Part model, mm, in its own coordinate system. Face numbers are marked on the shaded views. A direction names the side the tool comes from. Round coordinates to 2 decimals unless told otherwise and drop trailing zeros. Write each loop counter-clockwise with the first axis right and the second up, starting at its lowest first coordinate (ties: lowest second). Pieces come first, ordered by that corner, then holes. Notation, with made-up numbers: (3, 43.25) -> (28, 43.25) arc R18 ccw to (28, 62.25) -> close; hole circle Ø9 at (21, 54). An arc over 180 degrees is marked (long way). Use CSV: the item, a comma, the result in double quotes. Start each with the question number.
(1) Saw through at D-D (y = -47.5). Give the cut face in (x, z), plus the area to 3 significant figures.
(2) Which spindle directions (+Z, -Z, +X, -X, +Y, -Y) get a long thin tool onto all of the face, cutting with end or side? Do the marked faces 4, 5 and 6. Say none if no direction does.
(3) Probe line 1 (Z direction, x = -31, y = -28.25); line 2 (Z direction, x = -33, y = -42); line 3 (Z direction, x = -31, y = -26.75). List the from-to ranges inside material, lowest first. Write a range as [from, to].
(4) Saw through at C-C (x = 13). Give the cut face in (y, z), plus the area to 3 significant figures.
(5) Saw through at B-B (z = -27.5). Give the cut face in (x, y).
(6) Two-plate mould, pull along Y, no slides. Class the marked faces 1, 2 and 3: released by +Y, released by -Y, zero draft, split by the parting line, or undercut.
(7) Saw through at A-A (y = -25). Give the cut face in (x, z), plus the area to 3 significant figures.
(8) Drop flat-ended pins along their axis: pin 1 (8 mm diameter, centred on y = -8.5, z = -2, fed in from -X); pin 2 (18.5 mm diameter, centred on x = 7.5, y = -34.5, fed in from -Z); pin 3 (11.5 mm diameter, centred on x = -20, z = -8.5, fed in from -Y). Give the stop position or say it passes through.
```python
from build123d import *

# Parameters (mm, degrees)
EXTRUDE_1_DEPTH        = 5
FILLET_1_R             = 3
CUT_EXTRUDE_1_REACH    = 77
SKETCH_2_R             = 19.5
SKETCH_4_W             = 10
SKETCH_4_H             = 30
EXTRUDE_2_DEPTH        = 30
CUT_EXTRUDE_3_REACH    = 105.024
HOLE_WIZARD_M6_1_D     = 5
HOLE_WIZARD_M6_1_DEPTH = 15
HOLE_WIZARD_M6_1_TIP   = 1.502151548
SKETCH_7_W             = 55
SKETCH_7_H             = 10
EXTRUDE_3_DEPTH        = 12


with BuildPart() as part:
    # 草图1 → 凸台-拉伸1 (new, symmetric)
    with BuildSketch(Plane.XY):
        Polygon((0, 0), (55, 0), (55, -50), (-38, -50), (-38, -20), (0, -20), align=None)
    extrude(amount=EXTRUDE_1_DEPTH, both=True)

    # 圆角1
    fillet_1_edges = [part.edges().sort_by_distance(p)[0] for p in [
        (0, -20, 0),
    ]]
    fillet(fillet_1_edges, radius=FILLET_1_R)

    # 草图2 → 切除-拉伸1 (cut, up to next)
    with BuildSketch(Plane(origin=(0, 0, -5), x_dir=(-1, 0, 0), z_dir=(0, 0, -1)), mode=Mode.PRIVATE) as cut_extrude_1_sk1:
        with Locations((-25, -30)):
            Circle(SKETCH_2_R)
    cut_extrude_1_tool1 = extrude(cut_extrude_1_sk1.sketch, amount=-CUT_EXTRUDE_1_REACH, mode=Mode.PRIVATE) & part.part
    add(cut_extrude_1_tool1.solids().sort_by_distance((25, -30, -5))[0], mode=Mode.SUBTRACT)

    # 草图4 → 凸台-拉伸2 (add)
    with BuildSketch(Plane(origin=(0, 0, -5), x_dir=(-1, 0, 0), z_dir=(0, 0, -1))):
        with Locations((33, -35)):
            Rectangle(SKETCH_4_W, SKETCH_4_H)
    extrude(amount=EXTRUDE_2_DEPTH)

    # 草图5 → 切除-拉伸3 (cut, up to next)
    with BuildSketch(Plane(origin=(-28, 0, 0), x_dir=(0, 0, -1), z_dir=(1, 0, 0)), mode=Mode.PRIVATE) as cut_extrude_3_sk1:
        with BuildLine():
            Line((31, -27.5), (31, -42.5))
            ThreePointArc((31, -42.5), (27.5, -46), (24, -42.5))
            Line((24, -42.5), (24, -27.5))
            ThreePointArc((24, -27.5), (27.5, -24), (31, -27.5))
        make_face()
    cut_extrude_3_tool1 = extrude(cut_extrude_3_sk1.sketch, amount=-CUT_EXTRUDE_3_REACH, mode=Mode.PRIVATE) & part.part
    # 草图5 → 切除-拉伸3 (cut, up to next)
    with BuildSketch(Plane(origin=(-28, 0, 0), x_dir=(0, 0, -1), z_dir=(1, 0, 0)), mode=Mode.PRIVATE) as cut_extrude_3_sk2:
        with BuildLine():
            Line((19, -27.5), (19, -42.5))
            ThreePointArc((19, -42.5), (15.5, -46), (12, -42.5))
            Line((12, -42.5), (12, -27.5))
            ThreePointArc((12, -27.5), (15.5, -24), (19, -27.5))
        make_face()
    cut_extrude_3_tool2 = extrude(cut_extrude_3_sk2.sketch, amount=-CUT_EXTRUDE_3_REACH, mode=Mode.PRIVATE) & part.part
    add(cut_extrude_3_tool1.solids().sort_by_distance((-28, -35, -27.5))[0], mode=Mode.SUBTRACT)
    add(cut_extrude_3_tool2.solids().sort_by_distance((-28, -35, -15.5))[0], mode=Mode.SUBTRACT)

    # M6 螺纹孔1
    with Locations(Plane(origin=(-31, -20, -1), x_dir=(0, 0, 1), z_dir=(0, 1, 0))):
        with Locations((0, 0)):
            Hole(HOLE_WIZARD_M6_1_D / 2, depth=HOLE_WIZARD_M6_1_DEPTH)
            with Locations((0, 0, -(HOLE_WIZARD_M6_1_DEPTH + HOLE_WIZARD_M6_1_TIP / 2))):  # 118° drill point
                Cone(0, HOLE_WIZARD_M6_1_D / 2, HOLE_WIZARD_M6_1_TIP, mode=Mode.SUBTRACT)

    # 草图7 → 凸台-拉伸3 (add)
    with BuildSketch(Plane.XZ.offset(50)):
        with Locations((27.5, 0)):
            Rectangle(SKETCH_7_W, SKETCH_7_H)
    extrude(amount=EXTRUDE_3_DEPTH)


solid = part.part
```
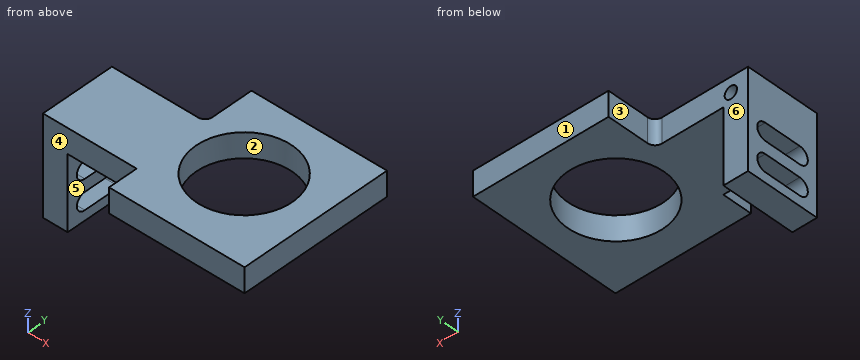
Answers:
1,outline,"(-38, -35) -> (-28, -35) -> (-28, -5) -> (16.4, -5) -> (16.4, 5) -> (-38, 5) -> close; (33.6, -5) -> (55, -5) -> (55, 5) -> (33.6, 5) -> close"
1,area,"1,060 mm²"
2,face 4,"+Z, -Z, -X, -Y"
2,face 5,"-Z, +X, +Y, -Y"
2,face 6,"+Z, -Z, -X, +Y"
3,line 1,"z = [-35, -31], [-24, -19], [-12, -3.5], [1.5, 5]"
3,line 2,"z = [-35, -31], [-24, -19], [-12, 5]"
3,line 3,"z = [-35, -30.92], [-24.08, -18.92], [-12.08, -3.5], [1.5, 5]"
4,outline,"(-62, -5) -> (-45.37, -5) -> (-45.37, 5) -> (-62, 5) -> close; (-14.63, -5) -> (0, -5) -> (0, 5) -> (-14.63, 5) -> close"
4,area,"313 mm²"
5,outline,"(-38, -50) -> (-28, -50) -> (-28, -46) -> (-38, -46) -> close; (-38, -24) -> (-28, -24) -> (-28, -20) -> (-38, -20) -> close"
6,face 1,"released by +Y"
6,face 2,"undercut"
6,face 3,"zero draft"
7,outline,"(-38, -35) -> (-28, -35) -> (-28, -29.95) -> (-38, -29.95) -> close; (-38, -25.05) -> (-28, -25.05) -> (-28, -17.95) -> (-38, -17.95) -> close; (-38, -13.05) -> (-28, -13.05) -> (-28, -5) -> (6.15, -5) -> (6.15, 5) -> (-38, 5) -> close; (43.85, -5) -> (55, -5) -> (55, 5) -> (43.85, 5) -> close; hole circle Ø5 at (-31, -1)"
7,area,"735 mm²"
8,pin 1,"stops at x = 0"
8,pin 2,"stops at z = -5"
8,pin 3,"stops at y = -50"
